from build123d import *

# Parameters (mm, degrees)
SKETCH_1_R      = 7.5
EXTRUDE_1_DEPTH = 22.5
CHAMFER_1_SIZE  = 0.5
SKETCH_4_W      = 0.5
SKETCH_4_H      = 1.2


with BuildPart() as part:
    # 草图1 → 凸台-拉伸1 (new, symmetric)
    with BuildSketch(Plane.XY):
        with Locations(Location((0, 0, 0), (0, 0, 180))):
            Circle(SKETCH_1_R)
    extrude(amount=EXTRUDE_1_DEPTH, both=True)

    # 草图2 → M8 螺纹孔1 (revolve, cut)
    with BuildSketch(Plane(origin=(0, 0, 22.5), x_dir=(0, -1, 0), z_dir=(1, 0, 0))):
        Polygon((0, 0), (0, 22.042926105), (3.4, 20), (3.4, 0), align=None)
    hole_wizard_m8_1 = revolve(axis=Axis((0, 0, 28.85), (0, 0, -1)), mode=Mode.SUBTRACT)

    # 倒角1
    chamfer_1_edges = [part.edges().sort_by_distance(p)[0] for p in [
        (7.5, 0, -22.5),
        (7.5, 0, 22.5),
    ]]
    chamfer(chamfer_1_edges, length=CHAMFER_1_SIZE)

    # 镜向3: M8 螺纹孔1 across plane
    add(hole_wizard_m8_1.mirror(Plane.XY), mode=Mode.SUBTRACT)

    # 草图4 → 切除-旋转1 (revolve, cut)
    with BuildSketch(Plane(origin=(0, 0, 0), x_dir=(1, 0, 0), z_dir=(0, 1, 0)), mode=Mode.PRIVATE) as cut_revolve_1_sk:
        with Locations((7.25, 15.1)):
            Rectangle(SKETCH_4_W, SKETCH_4_H)
    cut_revolve_1 = revolve(cut_revolve_1_sk.sketch.rotate(Axis((0, 0, -24.688510649), (0, 0, 1)), 180), axis=Axis((0, 0, -24.688510649), (0, 0, 1)), mode=Mode.SUBTRACT)

    # 镜向5: 切除-旋转1 across plane
    add(cut_revolve_1.mirror(Plane.XY), mode=Mode.SUBTRACT)


solid = part.part
Check sheet for the modelled part. Datum: model origin and axes. Units: mm. A direction names the side the tool comes from. Coordinates: 2 decimals unless noted, no trailing zeros. Write each loop counter-clockwise with the first axis right and the second up, starting at its lowest first coordinate (ties: lowest second). Pieces come first, ordered by that corner, then holes. Notation, with made-up numbers: M 66,86 L 93,86 A20 ccw 93,114 Z; hole C 88,-24.75 d4. An arc over 180 degrees is marked long. Answer as CSV lines item,"result".
Q1. Cross-section at A-A (z = 19). Record the boundary of the cut face in (x, y), then the cut area to 3 significant figures.
Check result:
outline,"C 0,0 d15; hole C 0,0 d6.8"
area,"140 mm^2"
Q2. Set-up check for faces 1 (the face through (-2, 7, 14.5)), 2 (the face through (-4.032, -6.324, 0.203)), 3 (the face through (3.32, 0.74, 12.64)): record each of +Z, -Z, +X, -X, +Y, -Y from which the full face is reachable in a straight line by a thin tool's end or side.
Check result:
face 1,"none"
face 2,"+Z, -Z"
face 3,"+Z"
Q3. Material ranges on probe 1 along Y at (x, z) = (0, 12.25); probe 2 along Y at (x, z) = (0, -15); probe 3 along Z at (x, y) = (5, -5.5), recorded low to high. Write a range as from..to.
Check result:
probe 1,"-7.5..-3.4, 3.4..7.5"
probe 2,"-7..-3.4, 3.4..7"
probe 3,"-22.07..-15.7, -14.5..14.5, 15.7..22.07"
Q4. Mould release check, pull along X, two halves, no side actions. Record for faces 4 (the face through (3.32, 0.74, -12.64)), 5 (the face through (-4.032, -6.324, -18.806)), 6 (the face through (-3, -2, -22.5)): released by +X, released by -X, zero draft, split by the parting line, or undercut.
Check result:
face 4,"undercut"
face 5,"split by the parting line"
face 6,"zero draft"
Q5. Go/stop test with flat-tipped pins: pin 1 (2 mm diameter, centred on x = 5.5, z = -17, fed in from -Y); pin 2 (5.5 mm diameter, centred on x = 0, y = 0, fed in from +Z); pin 3 (1.5 mm diameter, centred on y = 3.5, z = -15.5, fed in from -X). Record where each tip stops, or that it passes through.
Check result:
pin 1,"y = -6"
pin 2,"z = 2.11"
pin 3,"x = -6.97"
